```python
from build123d import *

# Parameters (mm, degrees)
SKETCH1_W           = 9
SKETCH1_H           = 6.5
BOSS_EXTRUDE1_DEPTH = 360
CHAMFER1_SIZE       = 0.3
SKETCH2_R           = 1.75
CUT_EXTRUDE1_DEPTH  = 37
LPATTERN1_COUNT     = 18
LPATTERN1_PITCH     = 20
SKETCH3_R           = 3
CUT_EXTRUDE2_DEPTH  = 4.5
LPATTERN2_COUNT     = 18
LPATTERN2_PITCH     = 20


with BuildPart() as part:
    # Sketch1 → Boss-Extrude1 (new body)
    with BuildSketch(Plane(origin=(0, 0, 0), x_dir=(1, 0, 0), z_dir=(0, 1, 0))):
        Rectangle(SKETCH1_W, SKETCH1_H)
    extrude(amount=BOSS_EXTRUDE1_DEPTH)

    # Chamfer1
    chamfer1_edges = [part.edges().sort_by_distance(p)[0] for p in [
        (-4.5, 180, -3.25),
        (4.5, 180, -3.25),
    ]]
    chamfer(chamfer1_edges, length=CHAMFER1_SIZE)

    # Sketch2 → Cut-Extrude1 (cut)
    with BuildSketch(Plane(origin=(0, 0, -3.25), x_dir=(-1, 0, 0), z_dir=(0, 0, -1))):
        with Locations((0, 10)):
            Circle(SKETCH2_R)
    cut_extrude1 = extrude(amount=-CUT_EXTRUDE1_DEPTH, mode=Mode.SUBTRACT)

    # LPattern1: Cut-Extrude1 ×18
    with Locations(*[(0, i * LPATTERN1_PITCH, 0) for i in range(1, LPATTERN1_COUNT)]):
        add(cut_extrude1, mode=Mode.SUBTRACT)

    # Sketch3 → Cut-Extrude2 (cut)
    with BuildSketch(Plane(origin=(0, 0, -3.25), x_dir=(-1, 0, 0), z_dir=(0, 0, -1))):
        with Locations((0, 10)):
            Circle(SKETCH3_R)
    cut_extrude2 = extrude(amount=-CUT_EXTRUDE2_DEPTH, mode=Mode.SUBTRACT)

    # LPattern2: Cut-Extrude2 ×18
    with Locations(*[(0, i * LPATTERN2_PITCH, 0) for i in range(1, LPATTERN2_COUNT)]):
        add(cut_extrude2, mode=Mode.SUBTRACT)


solid = part.part
```
The model under review builds one solid part; all positions refer to its coordinate system, in mm. Round coordinates to 2 decimals unless told otherwise and drop trailing zeros.
Item 1: To check wall thickness, follow probe 1 along X at (y, z) = (150, -1.6); probe 2 along X at (y, z) = (90, 2.05); probe 3 along Z at (x, y) = (4.25, 198). State the ranges of each line that lie inside material, in increasing order.
Working result:
probe 1: x = -4.5 to -3, 3 to 4.5
probe 2: x = -4.5 to -1.75, 1.75 to 4.5
probe 3: z = -3.2 to 3.25
Item 2: For pin 1 (1.5 mm diameter, centred on x = -1, z = -2.5, fed in from -Y); pin 2 (3 mm diameter, centred on x = 1, y = 151, fed in from -Z), all flat-tipped, find the tip position at first contact; note any pin that passes through.
Working result:
pin 1: stops at y = 0
pin 2: stops at z = 1.25
Item 3: Add section A-A, the plane x = 0. Count the separate pieces of the cut face and the enclosed holes in it, and give its area (3 significant figures).
Working result:
separate pieces: 19
enclosed holes: 0
area: 1,730 mm2
